from build123d import *

# Parameters (mm, degrees)
SKETCH_1_W              = 70
SKETCH_1_H              = 55
EXTRUDE_1_DEPTH         = 10
SKETCH_2_W              = 10
SKETCH_2_H              = 45
CUT_EXTRUDE_1_DEPTH     = 46.620718977
SKETCH_3_R              = 14
CUT_EXTRUDE_2_DEPTH     = 46.620718977
HOLE_WIZARD_M3_1_D      = 2.5
HOLE_WIZARD_5_5_5_5_1_D = 5.5
CHAMFER_1_SIZE          = 5
SKETCH_12_W             = 24
SKETCH_12_H             = 9
CUT_EXTRUDE_3_DEPTH     = 46.620718977
CHAMFER_2_SIZE          = 0.5


with BuildPart() as part:
    # 草图1 → 凸台-拉伸1 (new body)
    with BuildSketch(Plane.XY):
        Rectangle(SKETCH_1_W, SKETCH_1_H)
    extrude(amount=EXTRUDE_1_DEPTH)

    # 草图2 → 切除-拉伸1 (cut, through all)
    with BuildSketch(Plane.XY.offset(10)):
        with Locations((-30, -5)):
            Rectangle(SKETCH_2_W, SKETCH_2_H)
        with Locations((30, -5)):
            Rectangle(SKETCH_2_W, SKETCH_2_H)
    extrude(amount=-CUT_EXTRUDE_1_DEPTH, mode=Mode.SUBTRACT)

    # 草图3 → 切除-拉伸2 (cut, through all)
    with BuildSketch(Plane(origin=(0, 0, 0), x_dir=(-1, 0, 0), z_dir=(0, 0, -1))):
        with Locations((0, -6.5)):
            Circle(SKETCH_3_R)
    extrude(amount=-CUT_EXTRUDE_2_DEPTH, mode=Mode.SUBTRACT)

    # M3 螺纹孔1 (through all)
    with Locations(Plane.XY.offset(10)):
        with Locations((12.375, -18.875), (-12.375, -18.875), (-12.375, 5.875), (12.375, 5.875)):
            Hole(HOLE_WIZARD_M3_1_D / 2)

    # Ø5.5 (5.5) 直径孔1 (through all)
    with Locations(Plane(origin=(0, 17.5, 0), x_dir=(-1, 0, 0), z_dir=(0, -1, 0))):
        with Locations((-30, -5), (30, -5)):
            Hole(HOLE_WIZARD_5_5_5_5_1_D / 2)

    # 倒角1
    chamfer_1_edges = [part.edges().sort_by_distance(p)[0] for p in [
        (-25, -27.5, 5),
        (25, -27.5, 5),
    ]]
    chamfer(chamfer_1_edges, length=CHAMFER_1_SIZE)

    # 草图12 → 切除-拉伸3 (cut, through all)
    with BuildSketch(Plane.XY.offset(10)):
        with Locations((0, 23)):
            Rectangle(SKETCH_12_W, SKETCH_12_H)
    extrude(amount=-CUT_EXTRUDE_3_DEPTH, mode=Mode.SUBTRACT)

    # 倒角2
    chamfer_2_edges = [part.edges().sort_by_distance(p)[0] for p in [
        (-35, 22.5, 10),
        (0, 18.5, 10),
        (12, 23, 10),
        (-30, 17.5, 0),
        (-35, 17.5, 5),
        (-30, 17.5, 10),
        (35, 22.5, 0),
        (35, 22.5, 10),
        (25, -2.5, 0),
        (30, 17.5, 0),
        (35, 17.5, 5),
        (30, 17.5, 10),
        (25, -2.5, 10),
        (-35, 22.5, 0),
        (23.5, 27.5, 0),
        (23.5, 27.5, 10),
        (-35, 27.5, 5),
        (35, 27.5, 5),
        (-25, -2.5, 10),
        (-25, -2.5, 0),
        (0, -27.5, 10),
        (22.5, -25, 10),
        (-22.5, -25, 10),
        (0, -27.5, 0),
        (22.5, -25, 0),
        (-22.5, -25, 0),
        (-23.5, 27.5, 0),
        (-23.5, 27.5, 10),
        (-12, 23, 0),
        (12, 23, 0),
        (0, 18.5, 0),
        (-12, 23, 10),
    ]]
    chamfer(chamfer_2_edges, length=CHAMFER_2_SIZE)


solid = part.part
The listing builds one solid part. Answer for the finished solid, in the listing's coordinates (mm). A direction names the side the tool comes from. Give positions to 0.01 mm unless a question says otherwise; leave off trailing zeros. Write each loop counter-clockwise with the first axis right and the second up, starting at its lowest first coordinate (ties: lowest second). Pieces come first, ordered by that corner, then holes.
Item 1: Flat-ended cylindrical pins translate along their axes: P1, Ø3, axis at y = -5, z = 6, coming from the +X side; P2, Ø2.5, axis at y = -3, z = 6.5, coming from the -X side. Find the tip coordinate at first contact, or state that the pin passes through.
Item 2: Section A-A, the plane x = 0 is taken. Write down the section's boundary in (y, z), plus the area to 4 significant figures.
Item 3: Which of the six approach directions +Z, -Z, +X, -X, +Y, -Y give full straight-line access (tool end or side, diameter ignored) to faces 1 (the flat face through (-27.7, 17.5, 7.1)), 2 (the flat face through (25, -3, 5)), 3 (the flat face through (-12, 23, 5))?
Item 4: Section C-C, the plane z = 5 is taken. Count the separate pieces of the cut face and the enclosed holes in it, plus the area to 3 significant figures.
Item 5: Find the intervals of material crossed by line 1 along Y through (x, z) = (-8.5, 9); line 2 along Y through (x, z) = (11.5, 8); line 3 along Y through (x, z) = (0, 7), in increasing order.
Item 6: Section B-B, the plane y = 24.5 is taken. Write down the section's boundary in (x, z).
Item 7: Section D-D, the plane y = -6.5 is taken. Write down the section's boundary in (x, z), plus the area to 4 significant figures.
Item 8: Determine the mould class of faces 4 (the flat face through (7, 6, 0)), 5 (the flat face through (-22.5, -25, 5.1)), 6 (the flat face through (0, 18.5, 5)) for opening direction X: released by +X, released by -X, zero draft, split by the parting line, or undercut.
Completed:
1. P1: stops at x = 25
1. P2: stops at x = -25
2. outline: (-27.5, 0.5) - (-27, 0) - (-20.5, 0) - (-20.5, 10) - (-27, 10) - (-27.5, 9.5) - close; (7.5, 0) - (18, 0) - (18.5, 0.5) - (18.5, 9.5) - (18, 10) - (7.5, 10) - close
2. area: 179.5 mm2
3. face 1: +Z, -Z, -X, -Y
3. face 2: +Z, -Z, +X, -Y
3. face 3: +Z, -Z, +Y
4. separate pieces: 3
4. enclosed holes: 5
4. area: 1,960 mm2
5. line 1: y = -27.5 to -17.62, 4.62 to 18.5
5. line 2: y = -27.5 to -19.77, -17.98 to -14.48, 1.48 to 4.98, 6.77 to 18.5
5. line 3: y = -27.5 to -20.5, 7.5 to 18.5
6. outline: (-35, 0.5) - (-34.5, 0) - (-12.5, 0) - (-12, 0.5) - (-12, 9.5) - (-12.5, 10) - (-34.5, 10) - (-35, 9.5) - close; (12, 0.5) - (12.5, 0) - (34.5, 0) - (35, 0.5) - (35, 9.5) - (34.5, 10) - (12.5, 10) - (12, 9.5) - close; hole circle Ø5.5 at (-30, 5); hole circle Ø5.5 at (30, 5)
7. outline: (-25, 0.5) - (-24.5, 0) - (-14, 0) - (-14, 10) - (-24.5, 10) - (-25, 9.5) - close; (14, 0) - (24.5, 0) - (25, 0.5) - (25, 9.5) - (24.5, 10) - (14, 10) - close
7. area: 219.5 mm2
8. face 4: zero draft
8. face 5: released by -X
8. face 6: undercut
